Input: part model. Units: mm. Frame: model coordinates. Coordinates: 2 decimals unless noted, no trailing zeros. Write each question's results on one line, items separated by ' | '. Start each with the question number.
1. First-contact query: pin 1 (2 mm diameter, centred on y = 693, z = -18, fed in from -X); pin 2 (1.1 mm diameter, centred on y = 399.5, z = -17.5, fed in from +X); pin 3 (5 mm diameter, centred on x = 10.5, z = -4, fed in from -Y); pin 4 (1.1 mm diameter, centred on y = 647.5, z = -17.5, fed in from -X). Flat tips, straight axial feed; report the tip coordinate or a pass-through.
2. Section query A-A, the plane y = 654. Count the separate pieces of the cut face and the enclosed holes in it, and give its area (3 significant figures).
3. Ray query, probe 1 along Z at (x, y) = (6, 110); probe 2 along Z at (x, y) = (4.5, 921.5). Return the intervals inside material, ascending.
```python
from build123d import *

# Parameters (mm, degrees)
SKETCH16_R     = 3.4
SKETCH16_R_2   = 3
MEMBER_1_DEPTH = 1013


with BuildPart() as part:
    # Sketch16 → Member 1 (new body)
    with BuildSketch(Plane(origin=(0, 0, 0), x_dir=(-1, 0, 0), z_dir=(0, 1, 0))):
        with BuildLine():
            Line((-5.1, 20), (-5.1, 19.5))
            Line((-5.1, 19.5), (-4.1, 19.5))
            Line((-4.1, 19.5), (-4.1, 17))
            Line((-4.1, 17), (-6.1, 17))
            Line((-6.1, 17), (-6.1, 18))
            Line((-6.1, 18), (-10.3, 18))
            Line((-10.3, 18), (-10.3, 12))
            Line((-10.3, 12), (-6, 7.7))
            Line((-6, 7.7), (6, 7.7))
            Line((6, 7.7), (10.3, 12))
            Line((10.3, 12), (10.3, 18))
            Line((10.3, 18), (6.1, 18))
            Line((6.1, 18), (6.1, 17))
            Line((6.1, 17), (4.1, 17))
            Line((4.1, 17), (4.1, 19.5))
            Line((4.1, 19.5), (5.1, 19.5))
            Line((5.1, 19.5), (5.1, 20))
            Line((5.1, 20), (15.5, 20))
            ThreePointArc((15.5, 20), (18.681980515, 18.681980515), (20, 15.5))
            Line((20, 15.5), (20, 5.1))
            Line((20, 5.1), (19.5, 5.1))
            Line((19.5, 5.1), (19.5, 4.1))
            Line((19.5, 4.1), (17, 4.1))
            Line((17, 4.1), (17, 6.1))
            Line((17, 6.1), (18, 6.1))
            Line((18, 6.1), (18, 10.3))
            Line((18, 10.3), (12, 10.3))
            Line((12, 10.3), (7.7, 6))
            Line((7.7, 6), (7.7, -6))
            Line((7.7, -6), (12, -10.3))
            Line((12, -10.3), (18, -10.3))
            Line((18, -10.3), (18, -6.1))
            Line((18, -6.1), (17, -6.1))
            Line((17, -6.1), (17, -4.1))
            Line((17, -4.1), (19.5, -4.1))
            Line((19.5, -4.1), (19.5, -5.1))
            Line((19.5, -5.1), (20, -5.1))
            Line((20, -5.1), (20, -15.5))
            ThreePointArc((20, -15.5), (18.681980515, -18.681980515), (15.5, -20))
            Line((15.5, -20), (5.1, -20))
            Line((5.1, -20), (5.1, -19.5))
            Line((5.1, -19.5), (4.1, -19.5))
            Line((4.1, -19.5), (4.1, -17))
            Line((4.1, -17), (6.1, -17))
            Line((6.1, -17), (6.1, -18))
            Line((6.1, -18), (10.3, -18))
            Line((10.3, -18), (10.3, -12))
            Line((10.3, -12), (6, -7.7))
            Line((6, -7.7), (-6, -7.7))
            Line((-6, -7.7), (-10.3, -12))
            Line((-10.3, -12), (-10.3, -18))
            Line((-10.3, -18), (-6.1, -18))
            Line((-6.1, -18), (-6.1, -17))
            Line((-6.1, -17), (-4.1, -17))
            Line((-4.1, -17), (-4.1, -19.5))
            Line((-4.1, -19.5), (-5.1, -19.5))
            Line((-5.1, -19.5), (-5.1, -20))
            Line((-5.1, -20), (-15.5, -20))
            ThreePointArc((-15.5, -20), (-18.681980515, -18.681980515), (-20, -15.5))
            Line((-20, -15.5), (-20, -5.1))
            Line((-20, -5.1), (-19.5, -5.1))
            Line((-19.5, -5.1), (-19.5, -4.1))
            Line((-19.5, -4.1), (-17, -4.1))
            Line((-17, -4.1), (-17, -6.1))
            Line((-17, -6.1), (-18, -6.1))
            Line((-18, -6.1), (-18, -10.3))
            Line((-18, -10.3), (-12, -10.3))
            Line((-12, -10.3), (-7.7, -6))
            Line((-7.7, -6), (-7.7, 6))
            Line((-7.7, 6), (-12, 10.3))
            Line((-12, 10.3), (-18, 10.3))
            Line((-18, 10.3), (-18, 6.1))
            Line((-18, 6.1), (-17, 6.1))
            Line((-17, 6.1), (-17, 4.1))
            Line((-17, 4.1), (-19.5, 4.1))
            Line((-19.5, 4.1), (-19.5, 5.1))
            Line((-19.5, 5.1), (-20, 5.1))
            Line((-20, 5.1), (-20, 15.5))
            ThreePointArc((-20, 15.5), (-18.681980515, 18.681980515), (-15.5, 20))
            Line((-15.5, 20), (-5.1, 20))
        make_face()
        Circle(SKETCH16_R, mode=Mode.SUBTRACT)
        with Locations((-15.556349186, 15.556349186)):
            Circle(SKETCH16_R_2, mode=Mode.SUBTRACT)
        with Locations((15.556349186, 15.556349186)):
            Circle(SKETCH16_R_2, mode=Mode.SUBTRACT)
        with Locations((15.556349186, -15.556349186)):
            Circle(SKETCH16_R_2, mode=Mode.SUBTRACT)
        with Locations((-15.556349186, -15.556349186)):
            Circle(SKETCH16_R_2, mode=Mode.SUBTRACT)
    extrude(amount=MEMBER_1_DEPTH)


solid = part.part
```
Answer:
1) pin 1: x = -19.74 | pin 2: x = 19.76 | pin 3: through | pin 4: x = -19.76
2) separate pieces: 1 | enclosed holes: 5 | area: 605 mm^2
3) probe 1: -20 to -17, -7.7 to 7.7, 17 to 20 | probe 2: -19.5 to -17, -7.7 to 7.7, 17 to 19.5
